Could you check a few things on this drawing? It's one solid part, dimensions in mm from its lowest x, y, z. A direction names the side the tool comes from. Give positions to 0.01 mm unless a question says otherwise; leave off trailing zeros. Order: outer loops, then holes, each group sorted by start corner. A loop starts at its lowest first (then second) coordinate and runs counter-clockwise, first axis right, second up.
Item 1: I want a section at B-B, the plane z = 6.5. Write out the boundary of the cut face in (x, y).
Item 2: Which directions (+Z, -Z, +X, -X, +Y, -Y) give clear straight access to the entire face, cutting with the end or side of a thin tool? Please do the marked faces 1 and 2.
Item 3: I want a section at A-A, the plane x = 6.5. Write out the boundary of the cut face in (y, z).
Item 4: I want a section at D-D, the plane y = 9. Write out the boundary of the cut face in (x, z).
Item 5: I want a section at C-C, the plane y = 13.5. Write out the boundary of the cut face in (x, z).
Item 6: If I drill on line 1 along Z through (x, y) = (31.5, 2); line 2 along Z through (x, y) = (6.5, 13), over which ranges is the centre line in solid material (lowest first)?
Item 7: If we mould it in two halves opening along Z, with no side actions, what happens to the marked faces 3, 4, 5 and 6? For each: +Z half, -Z half, draft (parallel to the pull), parting line (faces both ways), or undercut.
Item 8: I'm going to push flat-ended pins straight in: pin 1 Ø1.8 at (x, z) = (6.5, 5) entering from +Y; pin 2 Ø2 at (x, z) = (31.5, 31.5) entering from +Y. Where does each tip first touch, or does it pass through?
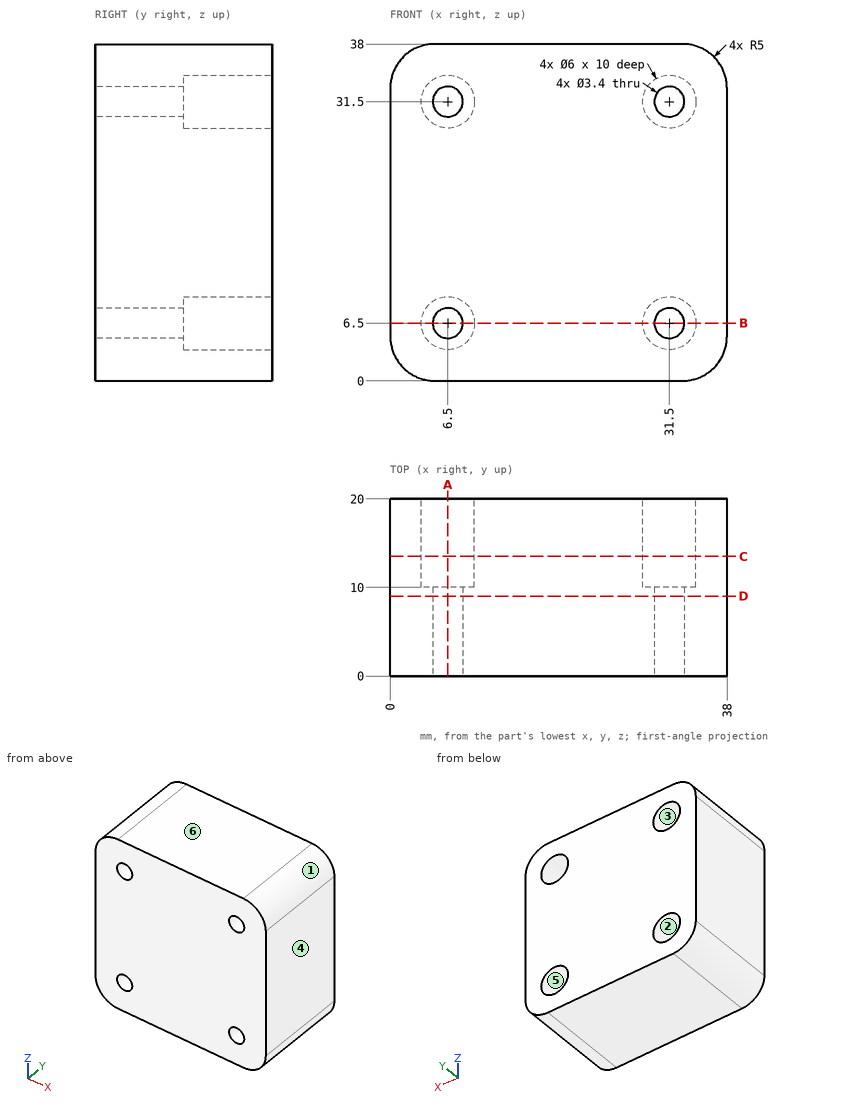
Results list:
1. outline: (0, 0) - (4.8, 0) - (4.8, 10) - (3.5, 10) - (3.5, 20) - (0, 20) - close; (8.2, 0) - (29.8, 0) - (29.8, 10) - (28.5, 10) - (28.5, 20) - (9.5, 20) - (9.5, 10) - (8.2, 10) - close; (33.2, 0) - (38, 0) - (38, 20) - (34.5, 20) - (34.5, 10) - (33.2, 10) - close
2. face 1: +Z, +X, +Y, -Y
2. face 2: +Y
3. outline: (0, 0) - (20, 0) - (20, 3.5) - (10, 3.5) - (10, 4.8) - (0, 4.8) - close; (0, 8.2) - (10, 8.2) - (10, 9.5) - (20, 9.5) - (20, 28.5) - (10, 28.5) - (10, 29.8) - (0, 29.8) - close; (0, 33.2) - (10, 33.2) - (10, 34.5) - (20, 34.5) - (20, 38) - (0, 38) - close
4. outline: (0, 5) arc R5 ccw to (5, 0) - (33, 0) arc R5 ccw to (38, 5) - (38, 33) arc R5 ccw to (33, 38) - (5, 38) arc R5 ccw to (0, 33) - close; hole circle Ø3.4 at (6.5, 6.5); hole circle Ø3.4 at (6.5, 31.5); hole circle Ø3.4 at (31.5, 6.5); hole circle Ø3.4 at (31.5, 31.5)
5. outline: (0, 5) arc R5 ccw to (5, 0) - (33, 0) arc R5 ccw to (38, 5) - (38, 33) arc R5 ccw to (33, 38) - (5, 38) arc R5 ccw to (0, 33) - close; hole circle Ø6 at (6.5, 6.5); hole circle Ø6 at (6.5, 31.5); hole circle Ø6 at (31.5, 6.5); hole circle Ø6 at (31.5, 31.5)
6. line 1: z = 0 to 4.8, 8.2 to 29.8, 33.2 to 38
6. line 2: z = 0 to 3.5, 9.5 to 28.5, 34.5 to 38
7. face 3: undercut
7. face 4: draft
7. face 5: undercut
7. face 6: +Z half
8. pin 1: stops at y = 10
8. pin 2: passes through
